Design review of the part built by this model. Coordinates are the model's own, in mm. Face numbers are marked on the shaded views. A direction names the side the tool comes from. Coordinates: 2 decimals unless noted, no trailing zeros. Write each loop counter-clockwise with the first axis right and the second up, starting at its lowest first coordinate (ties: lowest second). Pieces come first, ordered by that corner, then holes. Notation, with made-up numbers: (56.5, 87.25) - (103.5, 87.25) arc R28 ccw to (103.5, 113.25) - close; hole circle Ø7 at (66.25, -39). An arc over 180 degrees is marked (long way). Answer as CSV lines item,"result". Start each with the question number.
Q1. We need section A-A (z = 16). Write out the cut boundary in (x, y).
Q2. Machinability: for the marked faces 1, 2 and 3, which of the approach directions +Z, -Z, +X, -X, +Y, -Y give a long, thin tool a straight path to every point of the face, cutting with its end or side? Answer none if there is none.
Q3. Clearance check with flat-ended pins moving along their axes: pin 1 (3 mm diameter, centred on y = -28, z = 37, fed in from -X); pin 2 (6 mm diameter, centred on x = -56.5, z = 85, fed in from -Y); pin 3 (8 mm diameter, centred on y = -89, z = 22.5, fed in from -X). State where each tip first meets the part, or that it passes through.
Q4. For line 1 along Y through (x, z) = (0, 7); line 2 along Y through (x, z) = (-3, 84); line 3 along X through (y, z) = (2.5, 41.5), list the stretches that pass through material, from the lowest coordinate up. Write a range as [from, to].
from build123d import *

# Parameters (mm, degrees)
SKETCH_1_R             = 110
EXTRUDE_1_DEPTH        = 126
SKETCH_2_R             = 98
EXTRUDE_2_DEPTH        = 6
SKETCH_3_W             = 96
SKETCH_3_H             = 71.025255747
EXTRUDE_3_DEPTH        = 50
CHAMFER_1_SIZE         = 1
HOLE_WIZARD_M8_1_D     = 6.8
HOLE_WIZARD_M8_1_DEPTH = 19.75
HOLE_WIZARD_M8_1_TIP   = 2.042926105
HOLE_WIZARD_M8_2_D     = 6.8
HOLE_WIZARD_M8_2_DEPTH = 19.75
HOLE_WIZARD_M8_2_TIP   = 2.042926105


with BuildPart() as part:
    # 草图1 → 凸台-拉伸1 (new body)
    with BuildSketch(Plane.XY):
        Circle(SKETCH_1_R)
    extrude(amount=EXTRUDE_1_DEPTH)

    # 草图2 → 凸台-拉伸2 (add)
    with BuildSketch(Plane.XY.offset(126)):
        Circle(SKETCH_2_R)
    extrude(amount=EXTRUDE_2_DEPTH)

    # 草图3 → 凸台-拉伸3 (add)
    with BuildSketch(Plane(origin=(0, 0, 0), x_dir=(-1, 0, 0), z_dir=(0, 0, -1))):
        with Locations((0, -134.487372127)):
            Rectangle(SKETCH_3_W, SKETCH_3_H)
    extrude(amount=-EXTRUDE_3_DEPTH)

    # 倒角1
    chamfer_1_edges = [part.edges().sort_by_distance(p)[0] for p in [
        (-110, 0, 126),
        (-98, 0, 132),
    ]]
    chamfer(chamfer_1_edges, length=CHAMFER_1_SIZE)

    # M8 螺纹孔1
    with Locations(Plane(origin=(0, 0, 0), x_dir=(-1, 0, 0), z_dir=(0, 0, -1))):
        with Locations((0, 115), (81.317279836, 81.317279836), (115, 0), (81.317279836, -81.317279836), (0, -115), (-81.317279836, -81.317279836), (-115, 0), (-81.317279836, 81.317279836)):
            Hole(HOLE_WIZARD_M8_1_D / 2, depth=HOLE_WIZARD_M8_1_DEPTH)
            with Locations((0, 0, -(HOLE_WIZARD_M8_1_DEPTH + HOLE_WIZARD_M8_1_TIP / 2))):  # 118° drill point
                Cone(0, HOLE_WIZARD_M8_1_D / 2, HOLE_WIZARD_M8_1_TIP, mode=Mode.SUBTRACT)

    # M8 螺纹孔2
    with Locations(Plane.XY.offset(132)):
        with Locations((39.799076966, 96.083471381), (96.083471381, 39.799076966), (96.083471381, -39.799076966), (39.799076966, -96.083471381), (-39.799076966, -96.083471381), (-96.083471381, -39.799076966), (-96.083471381, 39.799076966), (-39.799076966, 96.083471381)):
            Hole(HOLE_WIZARD_M8_2_D / 2, depth=HOLE_WIZARD_M8_2_DEPTH)
            with Locations((0, 0, -(HOLE_WIZARD_M8_2_DEPTH + HOLE_WIZARD_M8_2_TIP / 2))):  # 118° drill point
                Cone(0, HOLE_WIZARD_M8_2_D / 2, HOLE_WIZARD_M8_2_TIP, mode=Mode.SUBTRACT)


solid = part.part
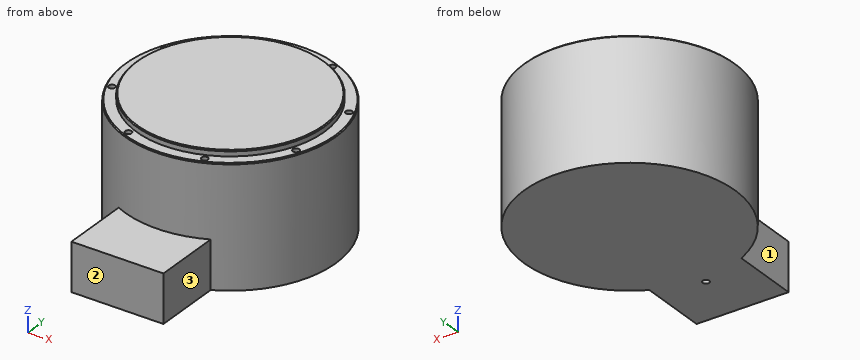
Results list:
1,outline,"(-48, -170) - (48, -170) - (48, -98.97) arc R110 ccw (long way) to (-48, -98.97) - close; hole circle Ø6.8 at (0, -115)"
2,face 1,"+Z, -Z, -X, -Y"
2,face 2,"+Z, -Z, +X, -X, -Y"
2,face 3,"+Z, -Z, +X, -Y"
3,pin 1,"stops at x = -106.76"
3,pin 2,"stops at y = -96.11"
3,pin 3,"stops at x = -69.82"
4,line 1,"y = [-170, -118.4], [-111.6, 110]"
4,line 2,"y = [-109.96, 109.96]"
4,line 3,"x = [-109.97, 109.97]"
